The figure shows three views and two pictorial views of one solid part (mm, origin at its lowest corner). Answer the questions. A direction names the side the tool comes from. Give positions to 0.01 mm unless a question says otherwise; leave off trailing zeros. Order: outer loops, then holes, each group sorted by start corner. A loop starts at its lowest first (then second) coordinate and runs counter-clockwise, first axis right, second up. Notation, with made-up numbers: (11.5, -9.5) - (47.5, -9.5) arc R24 cw to (47.5, 24.5) - close; hole circle Ø6 at (-8.5, -29.5). An arc over 180 degrees is marked (long way). Answer as a JSON object with one key per item and string values. Group by question number.
Q1. For the marked faces 1, 2 and 3, determine the directions among +Z, -Z, +X, -X, +Y, -Y from which every point of the face is accessible in a straight line to the end or side of a thin tool.
Q2. A cutting plane is placed at C-C, the plane y = 12.5. Give the vertices of the cut face in (x, z).
Q3. A cutting plane is placed at D-D, the plane y = 4.75. Give the vertices of the cut face in (x, z), and give its area (3 significant figures).
Q4. A cutting plane is placed at B-B, the plane z = 4.15. Give the vertices of the cut face in (x, y).
Q5. A cutting plane is placed at A-A, the plane x = 4.15. Give the vertices of the cut face in (y, z).
Q6. Given pin 1 (4 mm diameter, centred on y = 9, z = 7, fed in from -X); pin 2 (2 mm diameter, centred on x = 1.5, y = 3.5, fed in from +Z), each flat-ended and moving along its own axis, determine where each tip first touches the part or whether it passes through.
Q7. Consider line 1 (X direction, y = 12.5, z = 4.25); line 2 (Y direction, x = 2, z = 7.25); line 3 (Z direction, x = 6.25, y = 3.5). Determine where each line is inside the solid, lowest interval first.
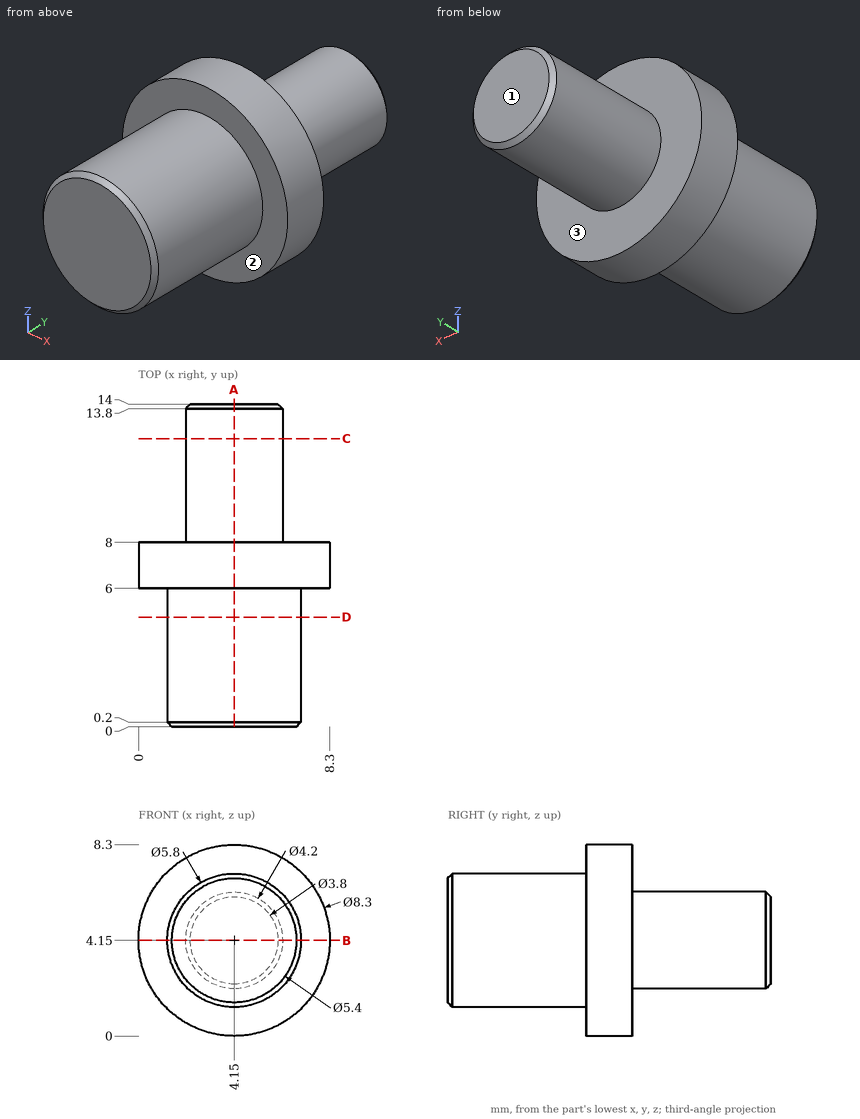
Reply:
{
 "1": {"face 1": "+Z, -Z, +X, -X, +Y", "face 2": "-Y", "face 3": "+Y"},
 "2": {"outline": "circle Ø4.2 at (4.15, 4.15)"},
 "3": {"outline": "circle Ø5.8 at (4.15, 4.15)", "area": "26.4 mm^2"},
 "4": {"outline": "(0, 6) - (1.25, 6) - (1.25, 0.2) - (1.45, 0) - (6.85, 0) - (7.05, 0.2) - (7.05, 6) - (8.3, 6) - (8.3, 8) - (6.25, 8) - (6.25, 13.8) - (6.05, 14) - (2.25, 14) - (2.05, 13.8) - (2.05, 8) - (0, 8) - close"},
 "5": {"outline": "(0, 1.45) - (0.2, 1.25) - (6, 1.25) - (6, 0) - (8, 0) - (8, 2.05) - (13.8, 2.05) - (14, 2.25) - (14, 6.05) - (13.8, 6.25) - (8, 6.25) - (8, 8.3) - (6, 8.3) - (6, 7.05) - (0.2, 7.05) - (0, 6.85) - close"},
 "6": {"pin 1": "stops at x = 0.15", "pin 2": "stops at z = 6.53"},
 "7": {"line 1": "x = 2.05 to 6.25", "line 2": "y = 6 to 8", "line 3": "z = 2.15 to 6.15"}
}
